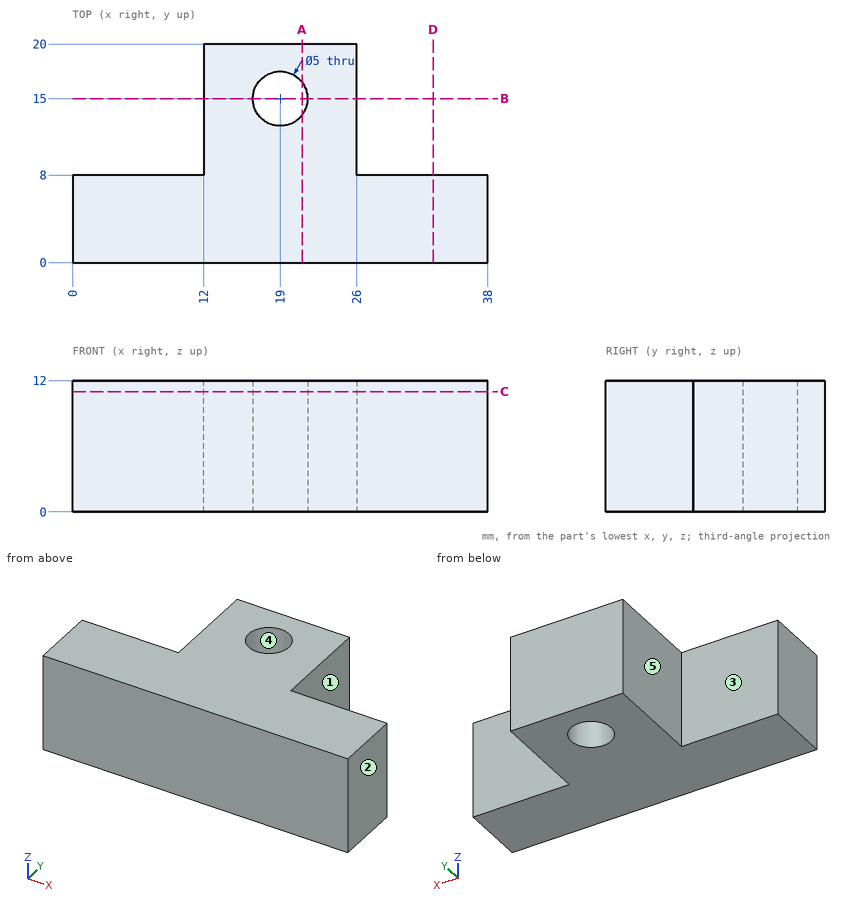
Design review of the part shown in the three views and the two pictorial views. Dimensions are in mm from the part's minimum x, y and z. A direction names the side the tool comes from. Round coordinates to 2 decimals unless told otherwise and drop trailing zeros. Loops run counter-clockwise (first coordinate to the right, second up) from the corner with the lowest first, then second, coordinate; pieces in that order, holes last. Notation, with made-up numbers: (22.5, 50.5) - (64.5, 50.5) arc R20 ccw to (64.5, 58.5) - close; hole circle Ø3 at (-3, -21.5). An arc over 180 degrees is marked (long way). Answer as CSV lines item,"result".
(1) Consider section A-A on x = 21. Give the boundary of the cut face in (y, z), then the cut area to 3 significant figures.
Checked values:
outline,"(0, 0) - (13.5, 0) - (13.5, 12) - (0, 12) - close; (16.5, 0) - (20, 0) - (20, 12) - (16.5, 12) - close"
area,"204 mm2"
(2) Consider section B-B on y = 15. Give the boundary of the cut face in (x, z), then the cut area to 3 significant figures.
Checked values:
outline,"(12, 0) - (16.5, 0) - (16.5, 12) - (12, 12) - close; (21.5, 0) - (26, 0) - (26, 12) - (21.5, 12) - close"
area,"108 mm2"
(3) Consider section C-C on z = 11. Give the boundary of the cut face in (x, y).
Checked values:
outline,"(0, 0) - (38, 0) - (38, 8) - (26, 8) - (26, 20) - (12, 20) - (12, 8) - (0, 8) - close; hole circle Ø5 at (19, 15)"
(4) Tool access review of the marked faces 1 and 2: name each direction out of +Z, -Z, +X, -X, +Y, -Y from which nothing blocks a thin tool from reaching the whole face with its end or side.
Checked values:
face 1,"+Z, -Z, +X, +Y"
face 2,"+Z, -Z, +X, +Y, -Y"
(5) Insertion check: P1, Ø6, axis at x = 34.5, z = 5.5, coming from the +Y side; P2, Ø6, axis at y = 12.5, z = 5, coming from the +X side. Each pin has a flat end and moves straight along its axis. Give the tip position at first contact, or say it passes through.
Checked values:
P1,"stops at y = 8"
P2,"stops at x = 26"
(6) Mouldability with a two-part tool opening along X and no side actions: class the marked faces 3, 4 and 5 as +X half, -X half, draft (parallel to the pull), parting line (faces both ways), or undercut.
Checked values:
face 3,"draft"
face 4,"undercut"
face 5,"-X half"
(7) Wall thickness on line 1 (Y direction, x = 19, z = 5.75); line 2 (Y direction, x = 29, z = 7.75); line 3 (X direction, y = 12, z = 1): over which ranges is each line inside the solid? List them lowest first.
Checked values:
line 1,"y = 0 to 12.5, 17.5 to 20"
line 2,"y = 0 to 8"
line 3,"x = 12 to 26"
(8) Consider section D-D on x = 33. Give the boundary of the cut face in (y, z).
Checked values:
outline,"(0, 0) - (8, 0) - (8, 12) - (0, 12) - close"
